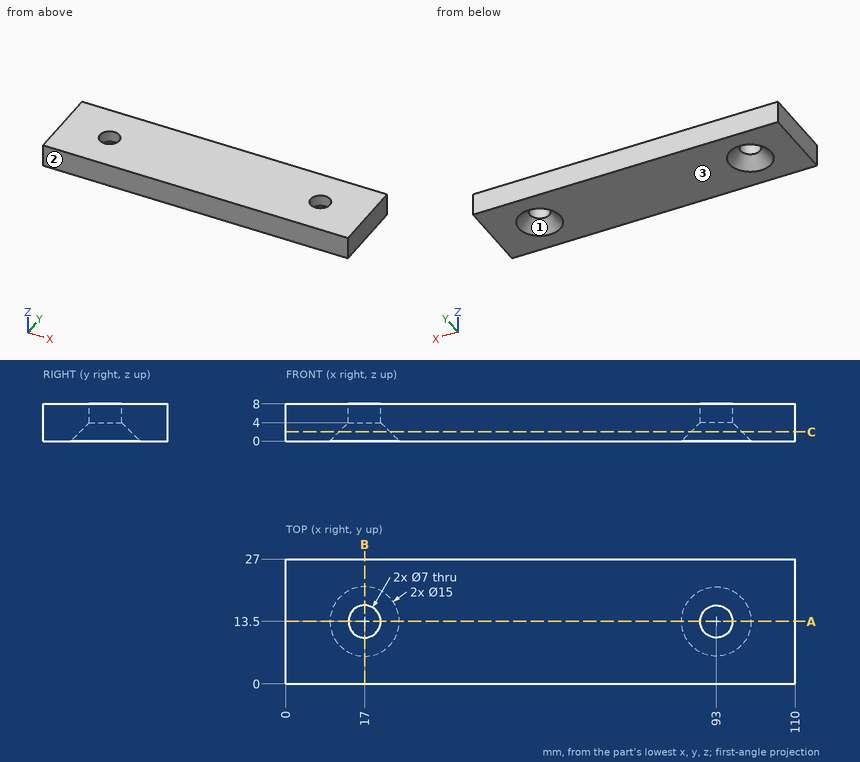
Study the drawing (mm; zero at the part's minimum x, y, z) and answer. Give positions to 0.01 mm unless a question says otherwise; leave off trailing zeros. Write each loop counter-clockwise with the first axis right and the second up, starting at its lowest first coordinate (ties: lowest second). Pieces come first, ordered by that corner, then holes.
(1) A flat-ended cylindrical pin translates along its axis: pin 1 Ø11 at (x, y) = (17, 13.5) entering from -Z. Find the tip coordinate at first contact, or state that the pin passes through.
Final values:
pin 1: stops at z = 2
(2) Straight lines are drawn through the part: line 1 (X direction, y = 13.5, z = 5); line 2 (Y direction, x = 93, z = 5.2); line 3 (X direction, y = 11, z = 1.5). For each, find the intervals that lie inside material, in ascending order.
Final values:
line 1: x = 0 to 13.5, 20.5 to 89.5, 96.5 to 110
line 2: y = 0 to 10, 17 to 27
line 3: x = 0 to 11.55, 22.45 to 87.55, 98.45 to 110
(3) The part is cut by section B-B on x = 17. Write down the section's boundary in (y, z).
Final values:
outline: (0, 0) - (6, 0) - (10, 4) - (10, 8) - (0, 8) - close; (17, 4) - (21, 0) - (27, 0) - (27, 8) - (17, 8) - close
(4) The mould has two halves that part along Y. Classify the marked faces 1, 2 and 3: pulls with the +Y half, pulls with the -Y half, needs draft (parallel to the pull), parting line crosses it, or undercut.
Final values:
face 1: undercut
face 2: pulls with the -Y half
face 3: needs draft
(5) The part is cut by section C-C on z = 2. Write down the section's boundary in (x, y).
Final values:
outline: (0, 0) - (110, 0) - (110, 27) - (0, 27) - close; hole circle Ø11 at (17, 13.5); hole circle Ø11 at (93, 13.5)
(6) The part is cut by section A-A on y = 13.5. Write down the section's boundary in (x, z).
Final values:
outline: (0, 0) - (9.5, 0) - (13.5, 4) - (13.5, 8) - (0, 8) - close; (20.5, 4) - (24.5, 0) - (85.5, 0) - (89.5, 4) - (89.5, 8) - (20.5, 8) - close; (96.5, 4) - (100.5, 0) - (110, 0) - (110, 8) - (96.5, 8) - close
